Could you check a few things on this model? Use its own coordinates, in mm. Round coordinates to 2 decimals unless told otherwise and drop trailing zeros. Loops run counter-clockwise (first coordinate to the right, second up) from the corner with the lowest first, then second, coordinate; pieces in that order, holes last.
from build123d import *

# Parameters (mm, degrees)
SKETCH1_R                  = 60
SKETCH1_R_2                = 32.5
BOSS_EXTRUDE1_DEPTH        = 34
F_13_0_13_DIAMETER_HOLE1_D = 13
CHAMFER1_SIZE              = 2


with BuildPart() as part:
    # Sketch1 → Boss-Extrude1 (new body)
    with BuildSketch(Plane.XY):
        Circle(SKETCH1_R)
        Circle(SKETCH1_R_2, mode=Mode.SUBTRACT)
    extrude(amount=BOSS_EXTRUDE1_DEPTH)

    # Ø13.0 (13) Diameter Hole1 (through all)
    with Locations(Plane(origin=(30.853778368, 51.459152348, 17), x_dir=(0.85765253914, -0.514229639467, 0), z_dir=(0.514229639467, 0.85765253914, 0))):
        with Locations((0, 0)):
            Hole(F_13_0_13_DIAMETER_HOLE1_D / 2)

    # Chamfer1
    chamfer1_edges = [part.edges().sort_by_distance(p)[0] for p in [
        (-60, 0, 0),
        (-60, 0, 34),
        (-32.5, 0, 0),
        (-32.5, 0, 34),
    ]]
    chamfer(chamfer1_edges, length=CHAMFER1_SIZE)


solid = part.part
Item 1: If we section it at A-A, the plane z = 13.5: Please give me the cut outline in (x, y), then the cut area to 3 significant figures.
Results list:
outline: (-35.42, -48.43) - (-21.17, -24.66) arc R32.5 cw to (11.78, 30.29) - (26.03, 54.06) arc R60 ccw to start; (-26.03, -54.06) arc R60 ccw to (35.42, 48.43) - (21.17, 24.66) arc R32.5 cw to (-11.78, -30.29) - close
area: 7,390 mm2
Item 2: If we section it at D-D, the plane z = 26.5: Please give me the cut outline in (x, y).
Results list:
outline: circle Ø120 at (0, 0); hole circle Ø65 at (0, 0)
Item 3: If I drill on line 1 along Y through (x, z) = (0, 22.5); line 2 along Y through (x, z) = (3.5, 17); line 3 along X through (y, z) = (18.5, 12), over which ranges is the centre line in solid material (lowest first)?
Results list:
line 1: y = -60 to -32.5, 32.5 to 60
line 2: y = -59.9 to -32.31, 32.31 to 59.9
line 3: x = -57.08 to -26.72, 26.72 to 57.08
Item 4: Will these pins go through, and if not, where does the flat tip stop? pin 1 (10 mm diameter, centred on y = 19.5, z = 19.5, fed in from -X); pin 2 (1.5 mm diameter, centred on y = 28, z = 18.5, fed in from +X) (3 decimals); pin 3 (1 mm diameter, centred on x = 22, z = 22.5, fed in from +Y); pin 4 (1.5 mm diameter, centred on x = 13, y = 42, fed in from -Z).
Results list:
pin 1: stops at x = -58.22
pin 2: stops at x = 53.455
pin 3: stops at y = 56.02
pin 4: stops at z = 0
Item 5: If we section it at B-B, the plane x = 0: Please give me the cut outline in (y, z), then the cut area to 3 significant figures.
Results list:
outline: (-60, 2) - (-58, 0) - (-34.5, 0) - (-32.5, 2) - (-32.5, 32) - (-34.5, 34) - (-58, 34) - (-60, 32) - close; (32.5, 2) - (34.5, 0) - (58, 0) - (60, 2) - (60, 32) - (58, 34) - (34.5, 34) - (32.5, 32) - close
area: 1,850 mm2
Item 6: We'd pull the mould along X, two halves only. Please class faces 1 (the flat face through (25, -25, 34)), 2 (the cylindrical face through (-18.15, -42.9, 16.71)), 3 (the cylindrical face through (-13.007, -58.573, 16.79)): released by +X, released by -X, zero draft, split by the parting line, or undercut.
Results list:
face 1: zero draft
face 2: undercut
face 3: split by the parting line
